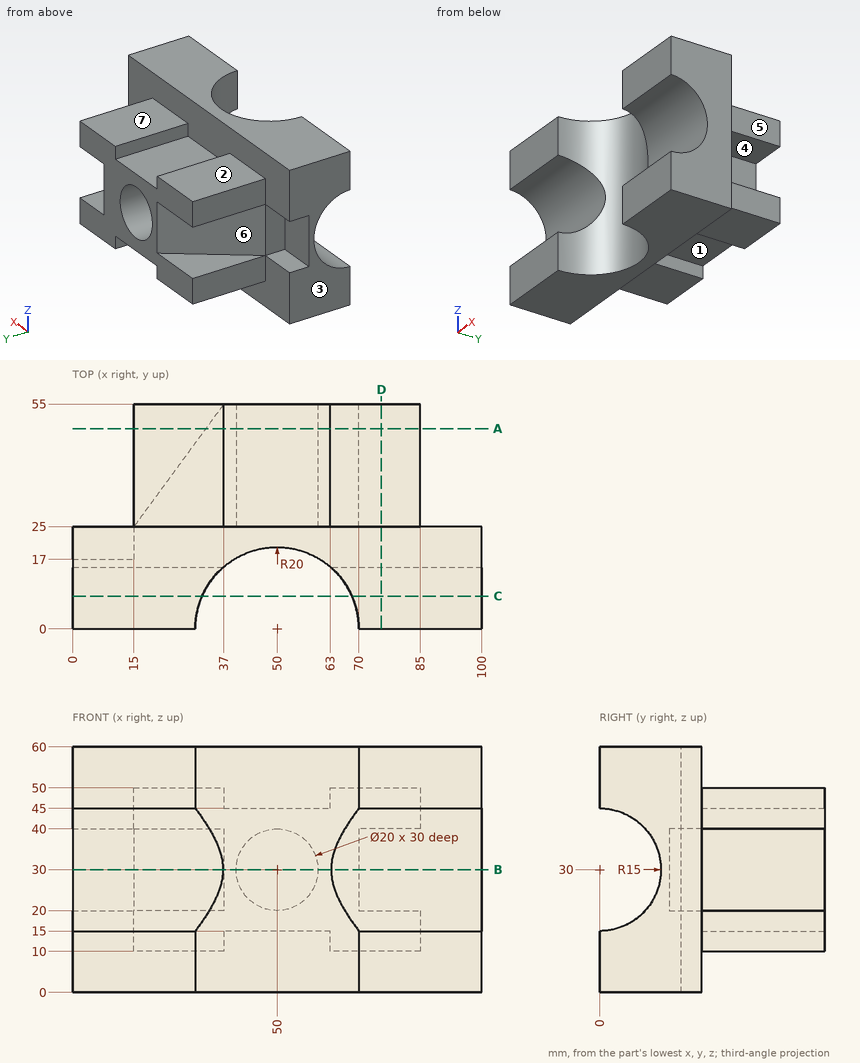
The figure shows three views and two pictorial views of one solid part (mm, origin at its lowest corner). Answer the questions. A direction names the side the tool comes from. Give positions to 0.01 mm unless a question says otherwise; leave off trailing zeros. Write each loop counter-clockwise with the first axis right and the second up, starting at its lowest first coordinate (ties: lowest second). Pieces come first, ordered by that corner, then holes. Notation, with made-up numbers: (-29.75, 1.25) - (27.25, 1.25) arc R13 ccw to (27.25, 20.25) - close; hole circle Ø6 at (15, -15). An arc over 180 degrees is marked (long way). Use one line per item in the form item = value.
1. A cutting plane is placed at C-C (y = 8). Write down the section's boundary in (x, z), and give its area (3 significant figures).
Filled in:
outline = (0, 0) - (31.67, 0) - (31.67, 17.31) - (0, 17.31) - close; (0, 42.69) - (31.67, 42.69) - (31.67, 60) - (0, 60) - close; (68.33, 0) - (100, 0) - (100, 17.31) - (68.33, 17.31) - close; (68.33, 42.69) - (100, 42.69) - (100, 60) - (68.33, 60) - close
area = 2,190 mm^2
2. A cutting plane is placed at D-D (x = 75.5). Write down the section's boundary in (y, z), and give its area (3 significant figures).
Filled in:
outline = (0, 0) - (25, 0) - (25, 10) - (55, 10) - (55, 20) - (25, 20) - (25, 40) - (55, 40) - (55, 50) - (25, 50) - (25, 60) - (0, 60) - (0, 45) arc R15 cw to (0, 15) - close
area = 1,750 mm^2
3. A cutting plane is placed at A-A (y = 49). Write down the section's boundary in (x, z), and give its area (3 significant figures).
Filled in:
outline = (15, 10) - (37, 10) - (37, 15) - (63, 15) - (63, 10) - (85, 10) - (85, 20) - (70, 20) - (70, 40) - (85, 40) - (85, 50) - (63, 50) - (63, 45) - (37, 45) - (37, 50) - (15, 50) - (15, 40) - (32.6, 40) - (32.6, 20) - (15, 20) - close; hole circle Ø20 at (50, 30)
area = 1,570 mm^2
4. Determine the mould class of the marked faces 1, 2 and 3 for opening direction X: released by +X, released by -X, zero draft, split by the parting line, or undercut.
Filled in:
face_1 = undercut
face_2 = zero draft
face_3 = released by -X
5. Each of these flat-tipped pins is pushed along its axis until it touches: pin 1 Ø4.5 at (x, z) = (5, 25.5) entering from +Y; pin 2 Ø11 at (y, z) = (34.5, 13.5) entering from +X; pin 3 Ø3 at (y, z) = (45.5, 13) entering from -X. Where does it stop, or does it pass through?
Filled in:
pin_1 = 17
pin_2 = 85
pin_3 = 15
6. Consider L1, parallel to X at y = 27, z = 12; L2, parallel to Z at x = 31, y = 47; L3, parallel to X at y = 24.5, z = 29. Determine where each line is inside the solid, lowest interval first.
Filled in:
L1 = 15 to 37, 63 to 85
L2 = 10 to 20, 40 to 50
L3 = 15 to 100
7. For the marked faces 4, 5, 6 and 7, determine the directions among +Z, -Z, +X, -X, +Y, -Y from which every point of the face is accessible in a straight line to the end or side of a thin tool.
Filled in:
face_4 = +X, +Y
face_5 = +Z, -Z, +X, +Y
face_6 = -X, +Y
face_7 = +Z, +X, -X, +Y
8. A cutting plane is placed at B-B (z = 30). Write down the section's boundary in (x, y).
Filled in:
outline = (0, 15) - (36.77, 15) arc R20 cw to (63.23, 15) - (100, 15) - (100, 25) - (70, 25) - (70, 55) - (60, 55) - (60, 25) - (40, 25) - (40, 55) - (37, 55) - (15, 25) - (15, 17) - (0, 17) - close
